Could you check a few things on this model? Use its own coordinates, in mm. A direction names the side the tool comes from. Coordinates: 2 decimals unless noted, no trailing zeros. Loops run counter-clockwise (first coordinate to the right, second up) from the corner with the lowest first, then second, coordinate; pieces in that order, holes last. Notation, with made-up numbers: (40.25, -15) - (76.25, -15) arc R22 cw to (76.25, 18) - close; hole circle Ø6 at (62.5, 69). An arc over 180 degrees is marked (long way). Put each result on its own line as item: value. Start each with the question number.
```python
from build123d import *

# Parameters (mm, degrees)
SKETCH1_R           = 4
BOSS_EXTRUDE1_DEPTH = 2
SKETCH3_R           = 2.975
BOSS_EXTRUDE2_DEPTH = 25
SKETCH4_R           = 2.85
BOSS_EXTRUDE3_DEPTH = 0.6
SKETCH5_R           = 2.975
BOSS_EXTRUDE4_DEPTH = 1.9
CHAMFER1_SIZE       = 0.5


with BuildPart() as part:
    # Sketch1 → Boss-Extrude1 (new body)
    with BuildSketch(Plane.XY):
        Circle(SKETCH1_R)
    extrude(amount=BOSS_EXTRUDE1_DEPTH)

    # Sketch3 → Boss-Extrude2 (add)
    with BuildSketch(Plane.XY.offset(2)):
        Circle(SKETCH3_R)
    extrude(amount=BOSS_EXTRUDE2_DEPTH)

    # Sketch4 → Boss-Extrude3 (add)
    with BuildSketch(Plane.XY.offset(27)):
        Circle(SKETCH4_R)
    extrude(amount=BOSS_EXTRUDE3_DEPTH)

    # Sketch5 → Boss-Extrude4 (add)
    with BuildSketch(Plane.XY.offset(27.6)):
        Circle(SKETCH5_R)
    extrude(amount=BOSS_EXTRUDE4_DEPTH)

    # Chamfer1
    chamfer1_edges = [part.edges().sort_by_distance(p)[0] for p in [
        (-2.975, 0, 29.5),
        (-4, 0, 0),
    ]]
    chamfer(chamfer1_edges, length=CHAMFER1_SIZE)


solid = part.part
```
(1) For pin 1 Ø4 at (x, z) = (-3, 26.5) entering from +Y; pin 2 Ø2 at (y, z) = (3, 25.5) entering from -X; pin 3 Ø3 at (y, z) = (-0.5, 5.5) entering from +X (3 decimals), each with a flat end and sliding along its axis, tell me the tip position at first contact or that it passes through.
(2) If we mould it in two halves opening along Z, with no side actions, what happens to faces 1 (the flat face through (0, 0, 0)), 2 (the cylindrical face through (-0.867, -3.905, 1.24)), 3 (the cylindrical face through (-2.262, -1.734, 27.296))? For each: pulls with the +Z half, pulls with the -Z half, needs draft (parallel to the pull), parting line crosses it, or undercut.
(3) I need wall thicknesses on L1, parallel to Y at x = 0, z = 9 (3 decimals); L2, parallel to Z at x = -2.75, y = 1.5; L3, parallel to Y at x = 2.25, z = 8.5. Which ranges of each line are inside material? Lowest first, please. Write a range as [from, to].
(4) I want a section at A-A on x = 0. List the corners of the cut face in (y, z) for me (3 decimals).
(5) I want a section at C-C on z = 19.25. List the corners of the cut face in (x, y) for me (3 decimals).
(6) Which directions (+Z, -Z, +X, -X, +Y, -Y) give clear straight access to the entire face, cutting with the end or side of a thin tool? Please do faces 4 (the flat face through (0, 0, 29.5)), 5 (the flat face through (-1, 3, 2)).
Answer sheet:
1. pin 1: stops at y = 2.8
1. pin 2: stops at x = -2.2
1. pin 3: stops at x = 2.975
2. face 1: pulls with the -Z half
2. face 2: needs draft
2. face 3: undercut
3. L1: y = [-2.975, 2.975]
3. L2: z = [0, 2]
3. L3: y = [-1.95, 1.95]
4. outline: (-4, 0.5) - (-3.5, 0) - (3.5, 0) - (4, 0.5) - (4, 2) - (2.975, 2) - (2.975, 27) - (2.85, 27) - (2.85, 27.6) - (2.975, 27.6) - (2.975, 29) - (2.475, 29.5) - (-2.475, 29.5) - (-2.975, 29) - (-2.975, 27.6) - (-2.85, 27.6) - (-2.85, 27) - (-2.975, 27) - (-2.975, 2) - (-4, 2) - close
5. outline: circle Ø5.95 at (0, 0)
6. face 4: +Z, +X, -X, +Y, -Y
6. face 5: +Z
